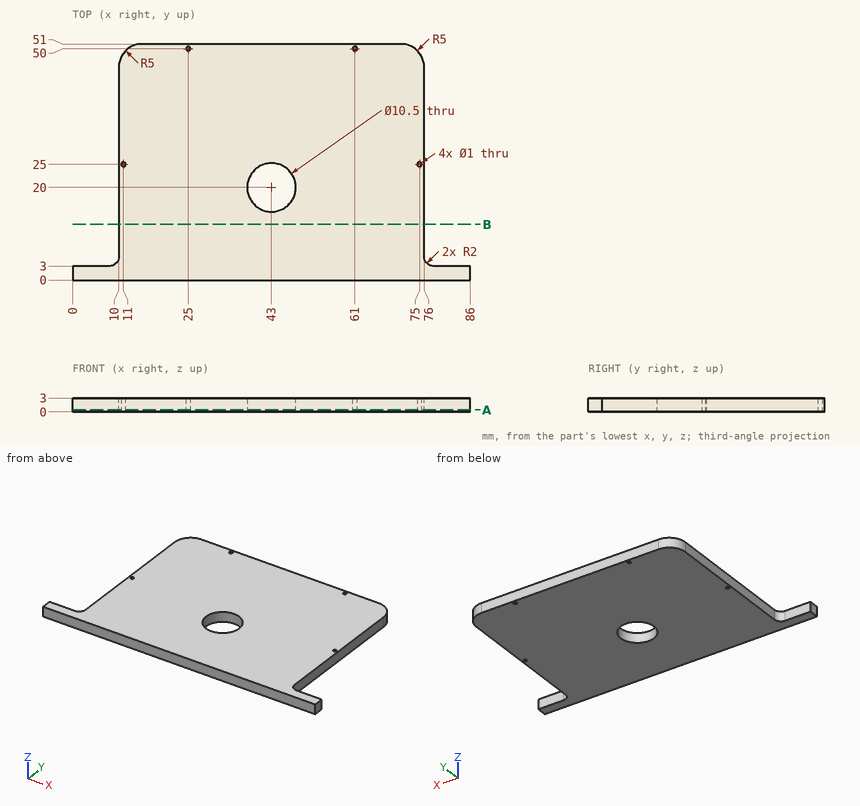
For this review, use the dimensioned drawing (mm, ordinates from the lowest corner) and the shaded views. Coordinates: 2 decimals unless noted, no trailing zeros. Write each loop counter-clockwise with the first axis right and the second up, starting at its lowest first coordinate (ties: lowest second). Pieces come first, ordered by that corner, then holes. Notation, with made-up numbers: (-3, 52) - (21, 52) arc R8 cw to (21, 65) - close; hole circle Ø6 at (46, -13). An arc over 180 degrees is marked (long way). One line per item, written item: value.
1) Insertion check: pin 1 (0.9 mm diameter, centred on x = 3.5, z = 1.5, fed in from +Y); pin 2 (1.5 mm diameter, centred on y = 26.5, z = 1, fed in from +X). Each pin has a flat end and moves straight along its axis. Give the tip position at first contact, or say it passes through.
Answer sheet:
pin 1: stops at y = 3
pin 2: stops at x = 76
2) To check wall thickness, follow probe 1 along Y at (x, z) = (43, 1); probe 2 along Y at (x, z) = (25, 2.15); probe 3 along X at (y, z) = (39, 1.9). State the ranges of each line that lie inside material, in increasing order.
Answer sheet:
probe 1: y = 0 to 14.75, 25.25 to 51
probe 2: y = 0 to 49.5, 50.5 to 51
probe 3: x = 10 to 76
3) Add section A-A (z = 0.45). State the section outline as (x, y) points, plus the area to 3 significant figures.
Answer sheet:
outline: (0, 0) - (86, 0) - (86, 3) - (78, 3) arc R2 cw to (76, 5) - (76, 46) arc R5 ccw to (71, 51) - (15, 51) arc R5 ccw to (10, 46) - (10, 5) arc R2 cw to (8, 3) - (0, 3) - close; hole circle Ø1 at (11, 25); hole circle Ø1 at (25, 50); hole circle Ø10.5 at (43, 20); hole circle Ø1 at (61, 50); hole circle Ø1 at (75, 25)
area: 3,330 mm2
4) Add section B-B (y = 12). State the section outline as (x, z) points, plus the area to 3 significant figures.
Answer sheet:
outline: (10, 0) - (76, 0) - (76, 3) - (10, 3) - close
area: 198 mm2
